Study the drawing (mm; zero at the part's minimum x, y, z) and answer. Give positions to 0.01 mm unless a question says otherwise; leave off trailing zeros. Order: outer loops, then holes, each group sorted by start corner. A loop starts at its lowest first (then second) coordinate and runs counter-clockwise, first axis right, second up.
Item 1: A cutting plane is placed at B-B (y = 2). Write down the section's boundary in (x, z), plus the area to 3 significant figures.
Item 2: A cutting plane is placed at C-C (x = 18.5). Write down the section's boundary in (y, z), plus the area to 3 significant figures.
Item 3: Given pin 1 Ø2 at (x, y) = (5.5, 4.5) entering from -Z, flat-ended and moving along its own axis, determine where the tip first touches the part or whether it passes through.
Item 4: Find the intervals of material crossed by line 1 along X through (y, z) = (1.75, 1.9); line 2 along X through (y, z) = (5.25, 3.9); line 3 along Y through (x, z) = (2.75, 5.1), in increasing order.
Item 5: A cutting plane is placed at A-A (z = 1.1). Write down the section's boundary in (x, y).
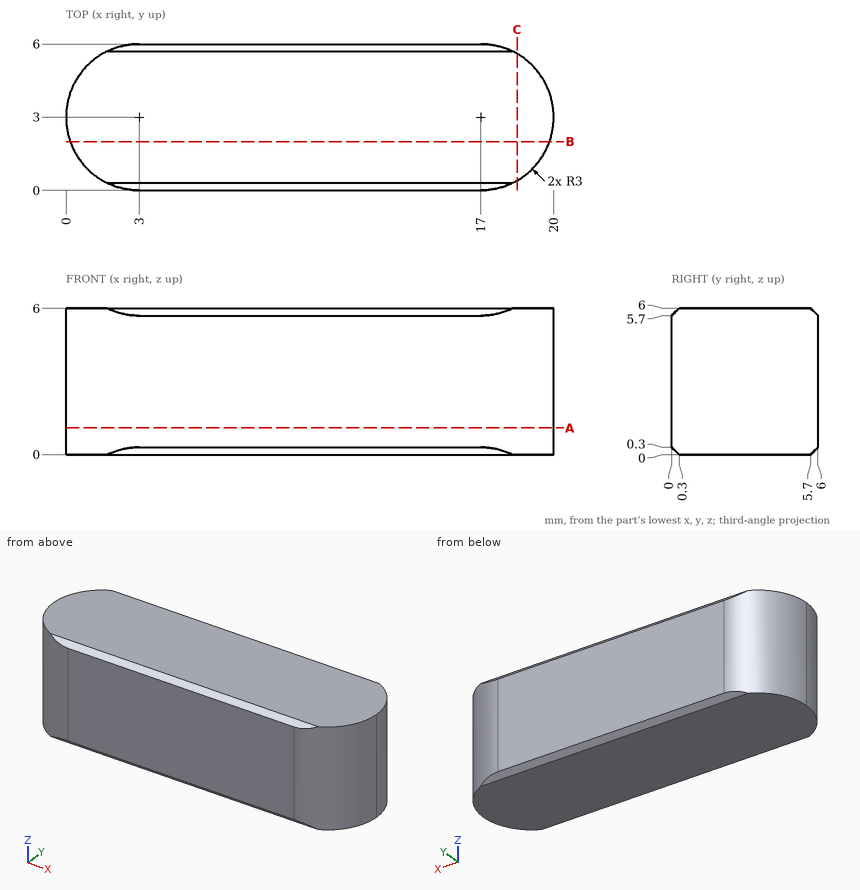
Response values:
1. outline: (0.17, 0) - (19.83, 0) - (19.83, 6) - (0.17, 6) - close
1. area: 118 mm2
2. outline: (0.4, 0) - (5.6, 0) - (5.6, 6) - (0.4, 6) - close
2. area: 31.2 mm2
3. pin 1: stops at z = 0
4. line 1: x = 0.27 to 19.73
4. line 2: x = 1.02 to 18.98
4. line 3: y = 0.01 to 5.99
5. outline: (3, 0) - (17, 0) arc R3 ccw to (17, 6) - (3, 6) arc R3 ccw to start
